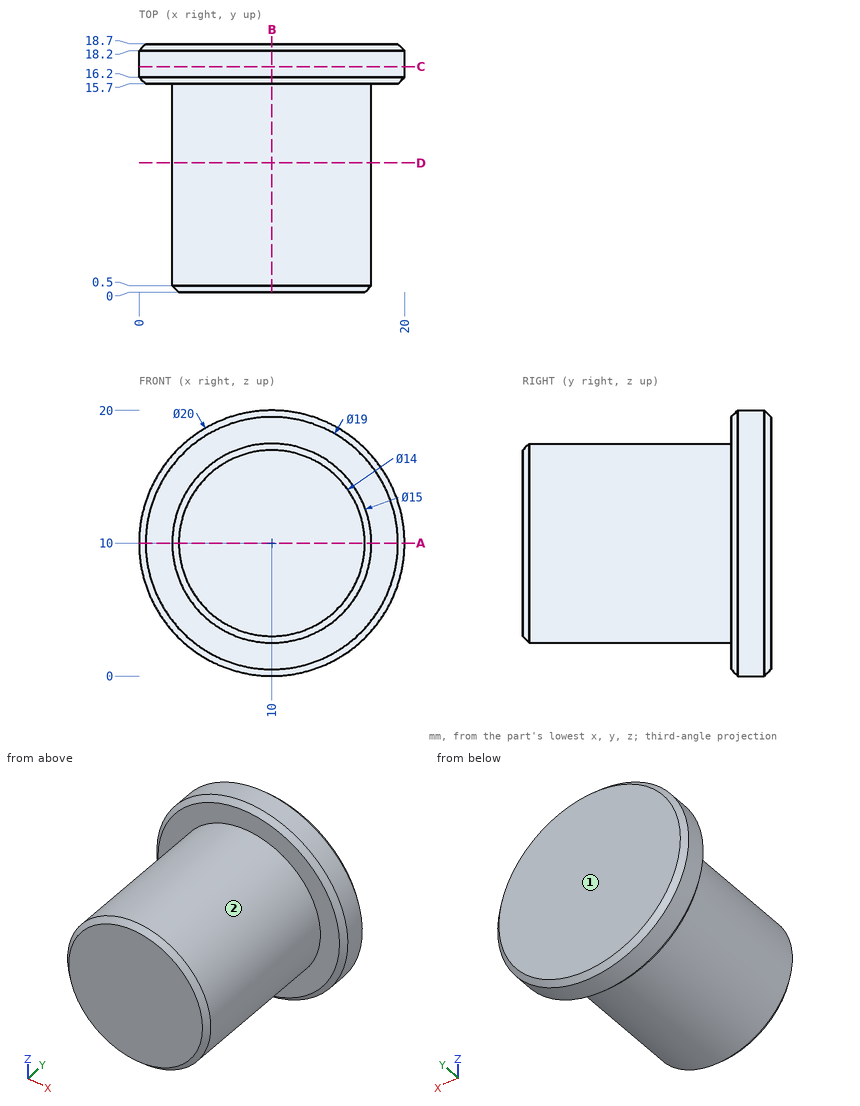
Input: dimensioned drawing with shaded views. Units: mm. Origin: part minimum x, y, z. A direction names the side the tool comes from. Round coordinates to 2 decimals unless told otherwise and drop trailing zeros. Loops run counter-clockwise (first coordinate to the right, second up) from the corner with the lowest first, then second, coordinate; pieces in that order, holes last. Notation, with made-up numbers: M 63.25,-6 L 84.25,-6 A19 cw 84.25,16 Z; hole C 83.5,28 d1. An arc over 180 degrees is marked long. Answer in a Markdown table with one row per item. Add a question column.
1. Section A-A (z = 10). Output: boundary loops of the cut face in (x, y), and give its area (3 significant figures).
2. Ray query, probe 1 along Y at (x, z) = (3.5, 14); probe 2 along Z at (x, y) = (18.75, 17.75); probe 3 along Z at (x, y) = (16.5, 13). Return the intervals inside material, ascending.
3. Contact query for flat-ended pins moving along their axis: pin 1 (4 mm diameter, centred on y = 14, z = 6.5, fed in from +X); pin 2 (1.5 mm diameter, centred on y = 10, z = 7, fed in from +X); pin 3 (1.5 mm diameter, centred on y = 8.5, z = 6.5, fed in from +X). Output: stop coordinate, or through.
4. Section D-D (y = 9.75). Output: boundary loops of the cut face in (x, z).
5. Section B-B (x = 10). Output: boundary loops of the cut face in (y, z).
6. Set-up query: the marked faces 1 and 2. Return all of +Z, -Z, +X, -X, +Y, -Y with unobstructed straight access to the full face (end or side cutting, diameter ignored); none if empty.
7. Section C-C (y = 17). Output: boundary loops of the cut face in (x, z).
Values follow:
| question | item | result |
|---|---|---|
| 1 | outline | M 0,16.2 L 0.5,15.7 L 2.5,15.7 L 2.5,0.5 L 3,0 L 17,0 L 17.5,0.5 L 17.5,15.7 L 19.5,15.7 L 20,16.2 L 20,18.2 L 19.5,18.7 L 0.5,18.7 L 0,18.2 Z |
| 1 | area | 295 mm^2 |
| 2 | probe 1 | 15.7 to 18.7 |
| 2 | probe 2 | 5.16 to 14.84 |
| 2 | probe 3 | 6.26 to 13.74 |
| 3 | pin 1 | x = 19.26 |
| 3 | pin 2 | x = 17.15 |
| 3 | pin 3 | x = 16.98 |
| 4 | outline | C 10,10 d15 |
| 5 | outline | M 0,3 L 0.5,2.5 L 15.7,2.5 L 15.7,0.5 L 16.2,0 L 18.2,0 L 18.7,0.5 L 18.7,19.5 L 18.2,20 L 16.2,20 L 15.7,19.5 L 15.7,17.5 L 0.5,17.5 L 0,17 Z |
| 6 | face 1 | +Z, -Z, +X, -X, +Y |
| 6 | face 2 | -Y |
| 7 | outline | C 10,10 d20 |
